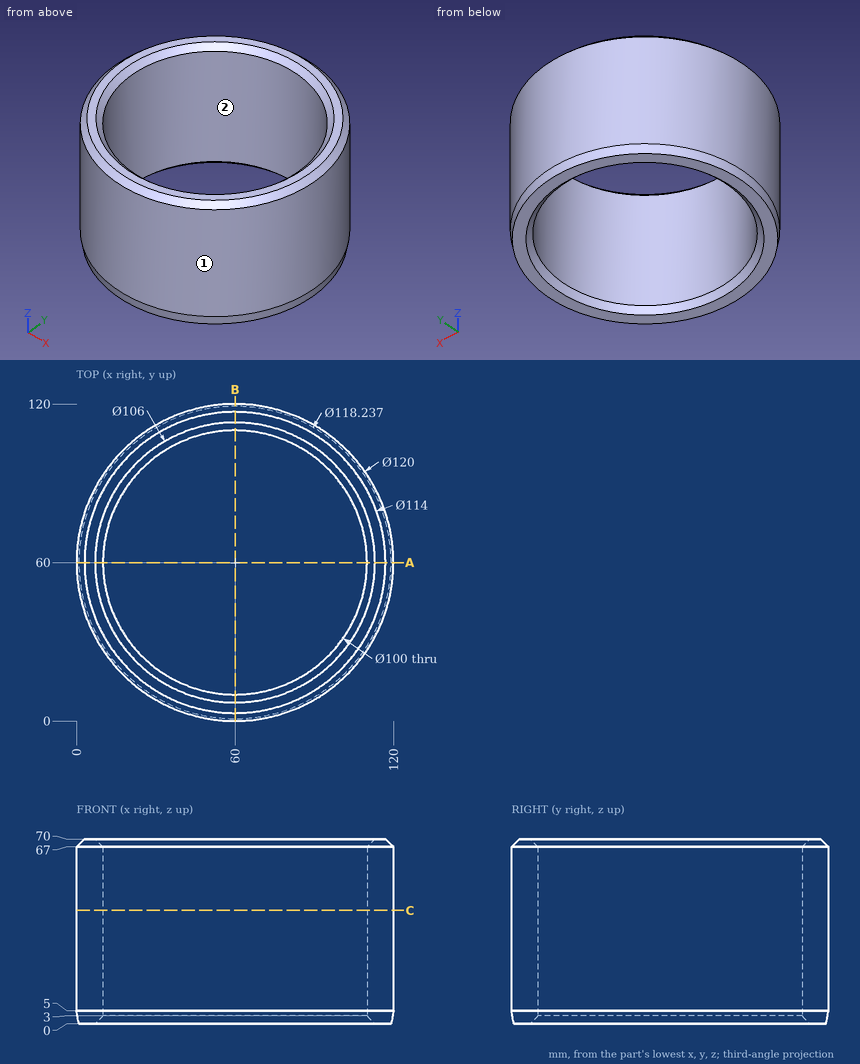
Could you check a few things on this drawing? It's one solid part, dimensions in mm from its lowest x, y, z. Give positions to 0.01 mm unless a question says otherwise; leave off trailing zeros. Order: outer loops, then holes, each group sorted by start corner. A loop starts at its lowest first (then second) coordinate and runs counter-clockwise, first axis right, second up. Notation, with made-up numbers: (-18, -27) -> (1, -27) arc R25 ccw to (1, 10) -> close; hole circle Ø9 at (-21.75, 72.25). An arc over 180 degrees is marked (long way). Use CSV: the item, a comma, the result in double quotes. Start each with the question number.
Item 1: Suppose I cut it at A-A (y = 60). List the corners of the cut face in (x, z) for me, and give its area (3 significant figures).
Item 2: I'm going to push flat-ended pins straight in: P1, Ø5, axis at x = 42, z = 54, coming from the +Y side; P2, Ø6, axis at y = 56, z = 53.5, coming from the -X side; P3, Ø6, axis at y = 103.5, z = 46, coming from the -X side. Where does each tip first touch, or does it pass through?
Item 3: Thinking about a two-plate mould opening in X: for the marked faces 1 and 2, which applies, pulls with the +X half, pulls with the -X half, needs draft (parallel to the pull), parting line crosses it, or undercut?
Item 4: Suppose I cut it at C-C (z = 43). List the corners of the cut face in (x, y) for me, and give its area (3 significant figures).
Item 5: If I drill on probe 1 along Y at (x, z) = (60, 52); probe 2 along Y at (x, z) = (84.5, 10.5) (1 decimal); probe 3 along X at (y, z) = (45.5, 4.5), over which ranges is the centre line in solid material (lowest first)? Write a range as [from, to].
Answer block:
1,outline,"(0, 5) -> (0.88, 0) -> (7, 0) -> (10, 3) -> (10, 67) -> (7, 70) -> (3, 70) -> (0, 67) -> close; (110, 3) -> (113, 0) -> (119.12, 0) -> (120, 5) -> (120, 67) -> (117, 70) -> (113, 70) -> (110, 67) -> close"
1,area,"1,370 mm^2"
2,P1,"stops at y = 117.96"
2,P2,"stops at x = 0.01"
2,P3,"stops at x = 15.73"
3,face 1,"parting line crosses it"
3,face 2,"undercut"
4,outline,"circle Ø120 at (60, 60); hole circle Ø100 at (60, 60)"
4,area,"3,460 mm^2"
5,probe 1,"y = [0, 10], [110, 120]"
5,probe 2,"y = [5.2, 16.4], [103.6, 114.8]"
5,probe 3,"x = [1.87, 12.15], [107.85, 118.13]"
